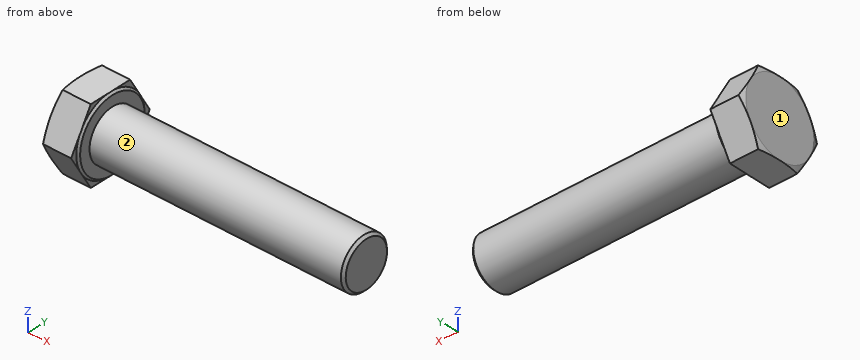
```python
from build123d import *

# Parameters (mm, degrees)
BASEHEAD_DEPTH = 12.715
SKETCH5_R      = 10
BASEBODY_DEPTH = 100
CHAMFER1_SIZE  = 1


with BuildPart() as part:
    # Sketch2 → BaseHead (new body)
    with BuildSketch(Plane(origin=(0, 0, 0), x_dir=(0, 0, -1), z_dir=(1, 0, 0))):
        Polygon((14.835, -8.564991243), (14.835, 8.564991243), (0, 17.129982487), (-14.835, 8.564991243), (-14.835, -8.564991243), (0, -17.129982487), align=None)
    extrude(amount=BASEHEAD_DEPTH)

    # Sketch3 → BearingFace (revolve, cut)
    with BuildSketch(Plane.XY, mode=Mode.PRIVATE) as bearingface_sk:
        Polygon((12.715, 17.129982487), (12.715, 14.095), (11.915, 14.895), (11.915, 17.129982487), align=None)
    revolve(bearingface_sk.sketch.rotate(Axis((-0.957090588, 0, 0), (1, 0, 0)), 90), axis=Axis((-0.957090588, 0, 0), (1, 0, 0)), mode=Mode.SUBTRACT)

    # Sketch4 → HeadChamfer (revolve, cut)
    with BuildSketch(Plane.XY):
        Polygon((0, 17.129982487), (0.835305313, 17.129982487), (0, 14.835), align=None)
    revolve(axis=Axis((-0.493528746, 0, 0), (1, 0, 0)), mode=Mode.SUBTRACT)

    # Sketch5 → BaseBody (add)
    with BuildSketch(Plane(origin=(12.715, 0, 0), x_dir=(0, 0, -1), z_dir=(1, 0, 0))):
        Circle(SKETCH5_R)
    extrude(amount=BASEBODY_DEPTH)

    # Chamfer1
    chamfer1_edges = [part.edges().sort_by_distance(p)[0] for p in [
        (112.715, 0, 10),
    ]]
    chamfer(chamfer1_edges, length=CHAMFER1_SIZE)


solid = part.part
```
Geometry: final body of the model. Coordinates: model frame, mm. Face numbers are marked on the shaded views. A direction names the side the tool comes from. Give positions to 0.01 mm unless a question says otherwise; leave off trailing zeros. Loops run counter-clockwise (first coordinate to the right, second up) from the corner with the lowest first, then second, coordinate; pieces in that order, holes last. Notation, with made-up numbers: (75, 80.5) -> (104, 80.5) arc R19 ccw to (104, 89.5) -> close; hole circle Ø4 at (31, -17.5). An arc over 180 degrees is marked (long way). Use CSV: the item, a comma, the result in double quotes.
(1) Ray query, line 1 along X through (y, z) = (1, 10) (3 decimals); line 2 along Z through (x, y) = (70.5, -3.5); line 3 along Z through (x, y) = (56.5, 9). Return the intervals inside material, ascending. Write a range as [from, to].
From the geometry:
line 1,"[0, 12.715]"
line 2,"[-9.37, 9.37]"
line 3,"[-4.36, 4.36]"
(2) Access query for the marked faces 1 and 2. Directions: +Z, -Z, +X, -X, +Y, -Y. A direction counts if a zero-diameter tool reaches every point of the face in a straight line with its end or side. Return the directions, or none.
From the geometry:
face 1,"+Z, -Z, -X, +Y, -Y"
face 2,"+X"
(3) Cut plane A-A (x = 99). Output: boundary loops of the cut face in (y, z).
From the geometry:
outline,"circle Ø20 at (0, 0)"
(4) First-contact query: P1, Ø3, axis at y = 15, z = -1.5, coming from the +X side (3 decimals); P2, Ø4, axis at x = 101, z = 9.5, coming from the -Y side; P3, Ø5, axis at y = -6, z = 10.5, coming from the +X side. Flat tips, straight axial feed; report the tip coordinate or a pass-through.
From the geometry:
P1,"x = 12.715"
P2,"y = -6.61"
P3,"x = 112.12"
